For this review, take the finished solid that the model builds, in its own axes (mm). A direction names the side the tool comes from. Round coordinates to 2 decimals unless told otherwise and drop trailing zeros. Order: outer loops, then holes, each group sorted by start corner. A loop starts at its lowest first (then second) coordinate and runs counter-clockwise, first axis right, second up. Notation, with made-up numbers: M 37.5,57 L 52.5,57 A11 ccw 52.5,78 Z; hole C 5.5,66.25 d7. An arc over 180 degrees is marked long. Put each result on its own line as item: value.
from build123d import *

# Parameters (mm, degrees)
CUT_EXTRUDE_3_DEPTH = 6
CUT_EXTRUDE_4_DEPTH = 7.3
CUT_EXTRUDE_5_DEPTH = 7.3


with BuildPart() as part:
    # 草图1 → 旋转1 (revolve)
    with BuildSketch(Plane(origin=(0, 0, 0), x_dir=(1, 0, 0), z_dir=(0, 1, 0))):
        Polygon((0, 100), (-12.5, 100), (-12.5, 74), (-25, 74), (-25, 38.53), (-27.5, 38.53), (-27.5, -387.93), (-25, -387.93), (-25, -422.93), (-12.5, -422.93), (-12.5, -448.93), (0, -448.93), align=None)
    revolve(axis=Axis((0, 0, 0), (0, 0, 1)))

    # 草图6 → 切除-拉伸3 (cut)
    with BuildSketch(Plane(origin=(0, 27.5, 0), x_dir=(1, 0, 0), z_dir=(0, 1, 0))):
        with BuildLine():
            Line((8, -131.93), (8, -175.93))
            ThreePointArc((8, -175.93), (0, -183.93), (-8, -175.93))
            Line((-8, -175.93), (-8, -131.93))
            ThreePointArc((-8, -131.93), (0, -123.93), (8, -131.93))
        make_face()
    extrude(amount=-CUT_EXTRUDE_3_DEPTH, mode=Mode.SUBTRACT)

    # 草图7 → 切除-拉伸4 (cut)
    with BuildSketch(Plane(origin=(14.434018231, -6.426438961, 0), x_dir=(0, 0, 1), z_dir=(-0.9135454576427331, 0.40673664307550317, 0))):
        with BuildLine():
            Line((-105.847779708, 4), (-83, 4))
            ThreePointArc((-83, 4), (-79, 0), (-83, -4))
            Line((-83, -4), (-105.847779708, -4))
            ThreePointArc((-105.847779708, -4), (-109.847779708, 0), (-105.847779708, 4))
        make_face()
    extrude(amount=CUT_EXTRUDE_4_DEPTH, mode=Mode.SUBTRACT)

    # 草图8 → 切除-拉伸5 (cut)
    with BuildSketch(Plane(origin=(6.426438961, 14.434018231, 0), x_dir=(0, 0, 1), z_dir=(-0.40673664307579893, -0.9135454576426014, 0))):
        with BuildLine():
            Line((455.303918894, -4), (431.93, -4))
            ThreePointArc((431.93, -4), (427.93, 0), (431.93, 4))
            Line((431.93, 4), (455.303918894, 4))
            ThreePointArc((455.303918894, 4), (459.303918894, 0), (455.303918894, -4))
        make_face()
    extrude(amount=CUT_EXTRUDE_5_DEPTH, mode=Mode.SUBTRACT)


solid = part.part
(1) Add section D-D on z = 400. Give the boundary of the cut face in (x, y).
A:
outline: C 0,0 d50
(2) Insertion check: pin 1 Ø1 at (x, y) = (13.5, -11) entering from +Z; pin 2 Ø8 at (x, z) = (-1, 141) entering from +Y; pin 3 Ø4 at (x, y) = (-14.5, 16) entering from -Z. Each pin has a flat end and moves straight along its axis. Give the tip position at first contact, or say it passes through.
A:
pin 1: stops at z = 422.93
pin 2: stops at y = 21.5
pin 3: stops at z = -74
(3) To check wall thickness, follow L1, parallel to Y at x = -2, z = 40; L2, parallel to Z at x = -11, y = -13; L3, parallel to X at y = -1.5, z = 379. State the ranges of each line that lie inside material, in increasing order.
A:
L1: y = -27.43 to 27.43
L2: z = -74 to 422.93
L3: x = -27.46 to 27.46
(4) Add section A-A on y = -19.5. Give the boundary of the cut face in (x, z).
A:
outline: M -19.39,-38.53 L -15.64,-38.53 L -15.64,-74 L 15.64,-74 L 15.64,-38.53 L 19.39,-38.53 L 19.39,387.93 L 15.64,387.93 L 15.64,422.93 L -15.64,422.93 L -15.64,387.93 L -19.39,387.93 Z
(5) For faces 1 (the face through (12.1, 22.3, -38.53)), 2 (the face through (0, 0, -100)), 3 (the face through (5.9, -11.5, 422.93)), list the 3-axis set-ups (+Z, -Z, +X, -X, +Y, -Y) from which the entire face can be reached by the end or side of a thin tool; tool diameter is ignored.
A:
face 1: -Z
face 2: -Z, +X, -X, +Y, -Y
face 3: +Z
(6) Add section B-B on z = 162. Give the boundary of the cut face in (x, y).
A:
outline: M -8,21.5 L -8,26.31 A27.5 ccw long 8,26.31 L 8,21.5 Z
(7) Add section C-C on z = 7. Give the boundary of the cut face in (x, y).
A:
outline: C 0,0 d55
(8) Draft analysis for pull direction Z (two halves, no side actions). For faces 4 (the face through (-23.846, -7.509, 405.675)), 5 (the face through (0, 21.5, 154)), 6 (the face through (-5.9, -11.5, -74)), state which applies: released by +Z, released by -Z, zero draft, split by the parting line, or undercut.
A:
face 4: zero draft
face 5: undercut
face 6: released by -Z
